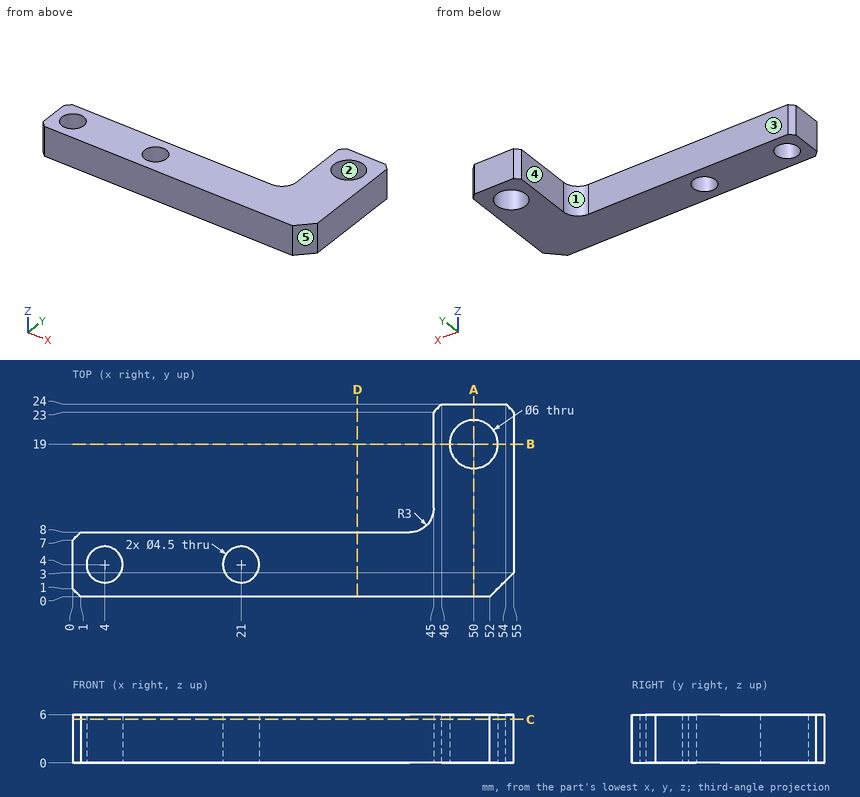
Can you work these out from the drawing? Everything is in mm from the part's minimum corner. A direction names the side the tool comes from. Coordinates: 2 decimals unless noted, no trailing zeros. Order: outer loops, then holes, each group sorted by start corner. A loop starts at its lowest first (then second) coordinate and runs counter-clockwise, first axis right, second up. Notation, with made-up numbers: M 52,66.5 L 68,66.5 A33 cw 68,100.5 Z; hole C 21.25,89.25 d8. An arc over 180 degrees is marked long. Answer as CSV lines item,"result". Start each with the question number.
1. I want a section at C-C, the plane z = 5.4. Write out the boundary of the cut face in (x, y), and give its area (3 significant figures).
2. For pin 1 (1.5 mm diameter, centred on y = 17.5, z = 4, fed in from -X); pin 2 (1.8 mm diameter, centred on x = 15.5, z = 4, fed in from +Y), each with a flat end and sliding along its axis, tell me the tip position at first contact or that it passes through.
3. On a 3-axis mill with a long thin cutter (end or side, diameter ignored), from which of +Z, -Z, +X, -X, +Y, -Y can I reach the whole of each face in a straight line? I mean the marked faces 4 and 5. Say none if no direction works.
4. We'd pull the mould along X, two halves only. Please class the marked faces 1, 2 and 3: released by +X, released by -X, zero draft, split by the parting line, or undercut.
5. I want a section at A-A, the plane x = 50. Write out the boundary of the cut face in (y, z), and give its area (3 significant figures).
6. I want a section at B-B, the plane y = 19. Write out the boundary of the cut face in (x, z), and give its area (3 significant figures).
7. I want a section at D-D, the plane x = 35.5. Write out the boundary of the cut face in (y, z).
8. I need wall thicknesses on line 1 (Y direction, x = 4, z = 1.2); line 2 (X direction, y = 3.5, z = 1.7); line 3 (Y direction, x = 12, z = 1.15). Which ranges of each line are inside material? Lowest first, please. Write a range as [from, to].
Recorded:
1,outline,"M 0,1 L 1,0 L 52,0 L 55,3 L 55,23 L 54,24 L 46,24 L 45,23 L 45,11 A3 cw 42,8 L 1,8 L 0,7 Z; hole C 4,4 d4.5; hole C 21,4 d4.5; hole C 50,19 d6"
1,area,"535 mm2"
2,pin 1,"stops at x = 45"
2,pin 2,"stops at y = 8"
3,face 4,"+Z, -Z, -X, +Y"
3,face 5,"+Z, -Z, +X, -Y"
4,face 1,"released by -X"
4,face 2,"undercut"
4,face 3,"zero draft"
5,outline,"M 0,0 L 16,0 L 16,6 L 0,6 Z; M 22,0 L 24,0 L 24,6 L 22,6 Z"
5,area,"108 mm2"
6,outline,"M 45,0 L 47,0 L 47,6 L 45,6 Z; M 53,0 L 55,0 L 55,6 L 53,6 Z"
6,area,"24.0 mm2"
7,outline,"M 0,0 L 8,0 L 8,6 L 0,6 Z"
8,line 1,"y = [0, 1.75], [6.25, 8]"
8,line 2,"x = [0, 1.81], [6.19, 18.81], [23.19, 55]"
8,line 3,"y = [0, 8]"
